The drawing under review shows one solid part. Ordinate dimensions are in mm from its lowest x, y, z. A direction names the side the tool comes from. Coordinates: 2 decimals unless noted, no trailing zeros. Order: outer loops, then holes, each group sorted by start corner. A loop starts at its lowest first (then second) coordinate and runs counter-clockwise, first axis right, second up.
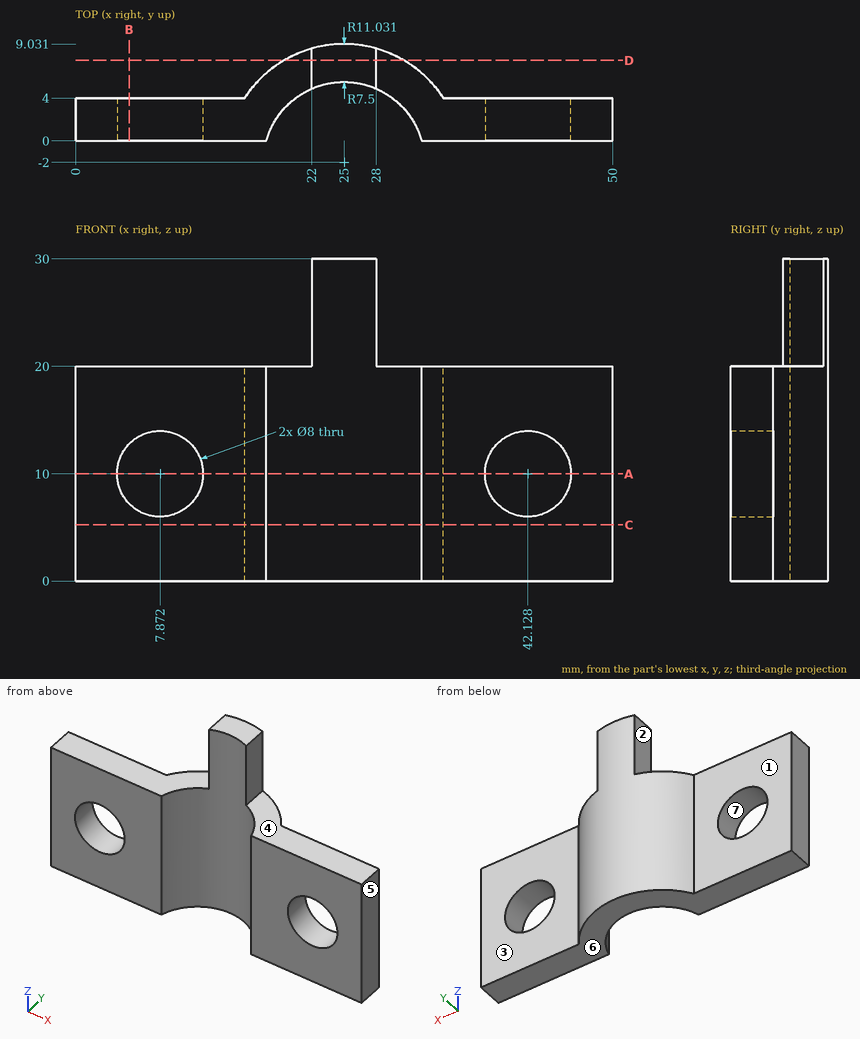
(1) We need section B-B, the plane x = 5. Write out the cut boundary in (y, z) (1 decimal).
A:
outline: (0, 0) - (4, 0) - (4, 7.2) - (0, 7.2) - close; (0, 12.8) - (4, 12.8) - (4, 20) - (0, 20) - close
(2) Wall thickness on probe 1 along Y at (x, z) = (8, 1.5); probe 2 along Z at (x, y) = (32.5, 4.75); probe 3 along Z at (x, y) = (39, 2.5) (1 decimal): over which ranges is each line inside the solid? List them lowest first.
A:
probe 1: y = 0 to 4
probe 2: z = 0 to 20
probe 3: z = 0 to 7.5, 12.5 to 20
(3) Draft analysis for pull direction Z (two halves, no side actions). For the marked faces 5, 6 and 7, state which applies: released by +Z, released by -Z, zero draft, split by the parting line, or undercut.
A:
face 5: zero draft
face 6: released by -Z
face 7: undercut
(4) We need section A-A, the plane z = 10. Write out the cut boundary in (x, y), and give its area (3 significant figures).
A:
outline: (0, 0) - (3.87, 0) - (3.87, 4) - (0, 4) - close; (11.87, 0) - (17.77, 0) arc R7.5 cw to (32.23, 0) - (38.13, 0) - (38.13, 4) - (34.26, 4) arc R11.03 ccw to (15.74, 4) - (11.87, 4) - close; (46.13, 0) - (50, 0) - (50, 4) - (46.13, 4) - close
area: 143 mm2
(5) We need section C-C, the plane z = 5.25. Write out the cut boundary in (x, y).
A:
outline: (0, 0) - (17.77, 0) arc R7.5 cw to (32.23, 0) - (50, 0) - (50, 4) - (34.26, 4) arc R11.03 ccw to (15.74, 4) - (0, 4) - close
(6) Machinability: for the marked faces 1, 2, 3 and 4, which of the approach directions +Z, -Z, +X, -X, +Y, -Y give a long, thin tool a straight path to every point of the face, cutting with its end or side? Answer none if there is none.
A:
face 1: +Z, -Z, -X, +Y
face 2: +Z, -X, +Y, -Y
face 3: +Z, -Z, +X, +Y
face 4: +Z, +X, +Y, -Y
(7) For pin 1 Ø10.5 at (x, z) = (7.87, 10) entering from -Y; pin 2 Ø4.5 at (x, y) = (34, 5.5) entering from +Z; pin 3 Ø8 at (x, z) = (6, 7) entering from +Y; pin 4 Ø4 at (y, z) = (6, 22.5) entering from +X, all flat-tipped, find the tip position at first contact; note any pin that passes through.
A:
pin 1: stops at y = 0
pin 2: stops at z = 20
pin 3: stops at y = 4
pin 4: stops at x = 28
(8) We need section D-D, the plane y = 7.5. Write out the cut boundary in (x, z), and give its area (3 significant figures).
A:
outline: (19.39, 0) - (30.61, 0) - (30.61, 20) - (28, 20) - (28, 30) - (22, 30) - (22, 20) - (19.39, 20) - close
area: 284 mm2
